from build123d import *

# Parameters (mm, degrees)
SKETCH_1_W          = 117
SKETCH_1_H          = 62
EXTRUDE_1_DEPTH     = 20
CUT_EXTRUDE_1_REACH = 71.161
SKETCH_2_R          = 21.5
SKETCH_3_W          = 43
SKETCH_3_H          = 31
CUT_EXTRUDE_2_DEPTH = 14
CHAMFER_1_SIZE      = 2


with BuildPart() as part:
    # 草图1 → 凸台-拉伸1 (new body)
    with BuildSketch(Plane.XY):
        Rectangle(SKETCH_1_W, SKETCH_1_H)
    extrude(amount=EXTRUDE_1_DEPTH)

    # 草图2 → 切除-拉伸1 (cut, up to next)
    with BuildSketch(Plane.XY.offset(20), mode=Mode.PRIVATE) as cut_extrude_1_sk1:
        Circle(SKETCH_2_R)
    cut_extrude_1_tool1 = extrude(cut_extrude_1_sk1.sketch, amount=-CUT_EXTRUDE_1_REACH, mode=Mode.PRIVATE) & part.part
    add(cut_extrude_1_tool1.solids().sort_by_distance((0, 0, 20))[0], mode=Mode.SUBTRACT)

    # 草图3 → 切除-拉伸2 (cut)
    with BuildSketch(Plane(origin=(0, 0, 0), x_dir=(-1, 0, 0), z_dir=(0, 0, -1))):
        with Locations((0, 15.5)):
            Rectangle(SKETCH_3_W, SKETCH_3_H)
    extrude(amount=-CUT_EXTRUDE_2_DEPTH, mode=Mode.SUBTRACT)

    # 倒角1
    chamfer_1_edges = [part.edges().sort_by_distance(p)[0] for p in [
        (0, 31, 14),
        (21.5, 31, 7),
        (-21.5, 31, 7),
    ]]
    chamfer(chamfer_1_edges, length=CHAMFER_1_SIZE)


solid = part.part
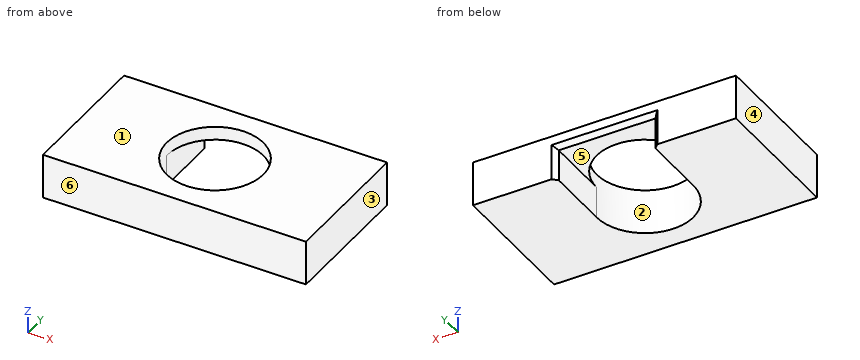
For this review, take the finished solid that the model builds, in its own axes (mm). Face numbers are marked on the shaded views. A direction names the side the tool comes from. Round coordinates to 2 decimals unless told otherwise and drop trailing zeros. Write each loop counter-clockwise with the first axis right and the second up, starting at its lowest first coordinate (ties: lowest second). Pieces come first, ordered by that corner, then holes. Notation, with made-up numbers: (85, -9.5) - (130, -9.5) arc R26 ccw to (130, 9.5) - close; hole circle Ø6 at (13, -27.5). An arc over 180 degrees is marked (long way). Use a Markdown table: item, result.
Q1. Machinability: for the marked faces 5 and 6, which of the approach directions +Z, -Z, +X, -X, +Y, -Y give a long, thin tool a straight path to every point of the face, cutting with its end or side? Answer none if there is none.
Derived:
| item | result |
|---|---|
| face 5 | -Z, +Y |
| face 6 | +Z, -Z, +X, -X, -Y |
Q2. We need section D-D (y = -8.5). Give the boundary of the cut face in (x, z), plus the area to 3 significant figures.
Derived:
| item | result |
|---|---|
| outline | (-58.5, 0) - (-19.75, 0) - (-19.75, 20) - (-58.5, 20) - close; (19.75, 0) - (58.5, 0) - (58.5, 20) - (19.75, 20) - close |
| area | 1,550 mm2 |
Q3. We need section C-C (z = 10.75). Give the boundary of the cut face in (x, y), plus the area to 3 significant figures.
Derived:
| item | result |
|---|---|
| outline | (-58.5, -31) - (58.5, -31) - (58.5, 31) - (23.5, 31) - (21.5, 29) - (21.5, 0) arc R21.5 cw to (-21.5, 0) - (-21.5, 29) - (-23.5, 31) - (-58.5, 31) - close |
| area | 5,190 mm2 |
Q4. The part is to be moulded in two halves that separate along X. For the marked faces 1, 2, 3 and 4, say which applies: pulls with the +X half, pulls with the -X half, needs draft (parallel to the pull), parting line crosses it, or undercut.
Derived:
| item | result |
|---|---|
| face 1 | needs draft |
| face 2 | undercut |
| face 3 | pulls with the +X half |
| face 4 | pulls with the -X half |
Q5. Wall thickness on line 1 along X through (y, z) = (0, 4.5); line 2 along Y through (x, z) = (0, 7.5); line 3 along Z through (x, y) = (2, 24): over which ranges is each line inside the solid? List them lowest first.
Derived:
| item | result |
|---|---|
| line 1 | x = -58.5 to -21.5, 21.5 to 58.5 |
| line 2 | y = -31 to -21.5 |
| line 3 | z = 14 to 20 |
Q6. Clearance check with a flat-ended pin moving along its axis: pin 1 (8 mm diameter, centred on x = -3, z = 2.5, fed in from +Y). State where the tip first meets the part, or that it passes through.
Derived:
| item | result |
|---|---|
| pin 1 | stops at y = -20.33 |
Q7. We need section A-A (x = 0). Give the boundary of the cut face in (y, z).
Derived:
| item | result |
|---|---|
| outline | (-31, 0) - (-21.5, 0) - (-21.5, 20) - (-31, 20) - close; (21.5, 14) - (29, 14) - (31, 16) - (31, 20) - (21.5, 20) - close |
Q8. We need section B-B (y = 18). Give the boundary of the cut face in (x, z).
Derived:
| item | result |
|---|---|
| outline | (-58.5, 0) - (-21.5, 0) - (-21.5, 14) - (-11.76, 14) - (-11.76, 20) - (-58.5, 20) - close; (11.76, 14) - (21.5, 14) - (21.5, 0) - (58.5, 0) - (58.5, 20) - (11.76, 20) - close |
